from build123d import *

# Parameters (mm, degrees)
BRACKET_PROFILE_SKETCH_R   = 13
BRACKET_PROFILE_SKETCH_R_2 = 20
BRACKET_PROFILE_SKETCH_R_3 = 10
BRACKET_PROFILE_SKETCH_R_4 = 22
BRACKET_PLATE_12_5MM_DEPTH = 12.5
EDGE_FILLET_R15_R          = 15


with BuildPart() as part:
    # Bracket Profile Sketch → Bracket Plate 12.5mm (new body)
    with BuildSketch(Plane.XY):
        with BuildLine():
            Line((0, 119.020008006), (0, 0))
            Line((0, 0), (44, 0))
            Line((44, 0), (44, 22))
            ThreePointArc((44, 22), (58, 36), (72, 22))
            Line((72, 22), (72, 0))
            Line((72, 0), (96, 0))
            Line((96, 0), (96, 70))
            ThreePointArc((96, 70), (91.01229045, 88.819901149), (77.358490566, 102.699370682))
            ThreePointArc((77.358490566, 102.699370682), (71.968832717, 108.178108656), (70, 115.607017004))
            Line((70, 115.607017004), (70, 170))
            ThreePointArc((70, 170), (86.946326412, 200.621771092), (52, 198.717797887))
            ThreePointArc((52, 198.717797887), (38.977494473, 183.164838251), (20, 176))
            ThreePointArc((20, 176), (-10.194037026, 154.598119083), (0, 119.020008006))
        make_face()
        with Locations((20, 22)):
            Circle(BRACKET_PROFILE_SKETCH_R, mode=Mode.SUBTRACT)
        with Locations((20, 144)):
            Circle(BRACKET_PROFILE_SKETCH_R_2, mode=Mode.SUBTRACT)
        with Locations((70, 190)):
            Circle(BRACKET_PROFILE_SKETCH_R_3, mode=Mode.SUBTRACT)
        with Locations((58, 70)):
            Circle(BRACKET_PROFILE_SKETCH_R_4, mode=Mode.SUBTRACT)
    extrude(amount=BRACKET_PLATE_12_5MM_DEPTH)

    # Edge Fillet R15
    edge_fillet_r15_edges = [part.edges().sort_by_distance(p)[0] for p in [
        (70, 170, 6.25),
    ]]
    fillet(edge_fillet_r15_edges, radius=EDGE_FILLET_R15_R)


solid = part.part
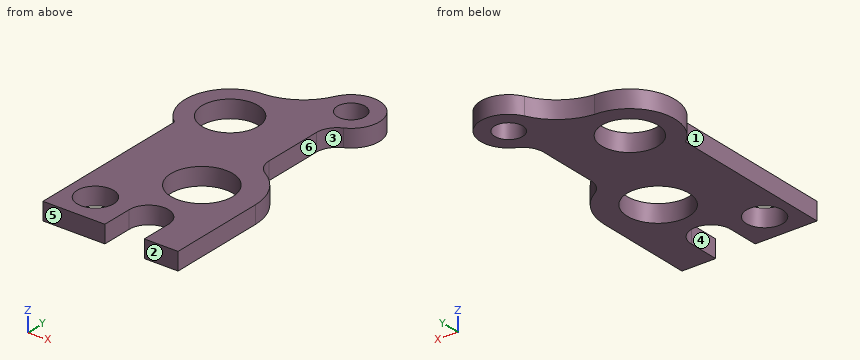
The model under review builds one solid part; all positions refer to its coordinate system, in mm. Face numbers are marked on the shaded views. A direction names the side the tool comes from. Give positions to 0.01 mm unless a question says otherwise; leave off trailing zeros. Order: outer loops, then holes, each group sorted by start corner. A loop starts at its lowest first (then second) coordinate and runs counter-clockwise, first axis right, second up. Notation, with made-up numbers: M 49,87 L 97,87 A9 ccw 97,99 Z; hole C -24,56 d2. An arc over 180 degrees is marked long. Answer in a Markdown table with one row per item. Add a question column.
1. Add section D-D on x = 24.5. State the section outline as (y, z) points.
2. Machinability: for the marked faces 4, 5 and 6, which of the approach directions +Z, -Z, +X, -X, +Y, -Y give a long, thin tool a straight path to every point of the face, cutting with its end or side? Answer none if there is none.
3. Mouldability with a two-part tool opening along Y and no side actions: class the marked faces 1, 2 and 3 as released by +Y, released by -Y, zero draft, split by the parting line, or undercut.
4. Add section C-C on x = 46.5. State the section outline as (y, z) points (3 decimals).
5. To check wall thickness, follow line 1 along Y through (x, z) = (20, 5.25); line 2 along Y through (x, z) = (29.5, 6.5); line 3 along X through (y, z) = (79, 6.75). State the ranges of each line that lie inside material, in increasing order.
6. Add section A-A on z = 5.75. State the section outline as (x, y) points, plus the area to 3 significant figures.
7. For pin 1 Ø6 at (y, z) = (130, 7.5) entering from +X; pin 2 Ø4 at (y, z) = (37, 10.5) entering from -X, all flat-tipped, find the tip position at first contact; note any pin that passes through.
8. Add section B-B on y = 144. State the section outline as (x, z) points, plus the area to 3 significant figures.
The answers:
| question | item | result |
|---|---|---|
| 1 | outline | M 0,0 L 9.8,0 L 9.8,12.5 L 0,12.5 Z; M 34.2,0 L 124.51,0 L 124.51,12.5 L 34.2,12.5 Z; M 163.49,0 L 176.73,0 L 176.73,12.5 L 163.49,12.5 Z |
| 2 | face 4 | +Z, -Z, -Y |
| 2 | face 5 | +Z, -Z, +X, -X, -Y |
| 2 | face 6 | +Z, -Z, +X |
| 3 | face 1 | zero draft |
| 3 | face 2 | released by -Y |
| 3 | face 3 | undercut |
| 4 | outline | M 29.984,0 L 51.245,0 L 51.245,12.5 L 29.984,12.5 Z; M 88.755,0 L 190.113,0 L 190.113,12.5 L 88.755,12.5 Z |
| 5 | line 1 | 0 to 9, 35 to 124, 164 to 176 |
| 5 | line 2 | 0 to 13.13, 30.87 to 126.4, 161.6 to 178.19 |
| 5 | line 3 | 0 to 37.93, 78.07 to 94.92 |
| 6 | outline | M 0,0 L 44,0 L 44,22 A14 cw 72,22 L 72,0 L 96,0 L 96,70 A38 ccw 77.36,102.7 A15 cw 70,115.61 L 70,158.38 A15 cw 78.57,171.93 A20 ccw long 52,198.72 A40 cw 20,176 A32 ccw 0,119.02 Z; hole C 20,144 d40; hole C 20,22 d26; hole C 58,70 d44; hole C 70,190 d20 |
| 6 | area | 12,100 mm2 |
| 7 | pin 1 | x = 70 |
| 7 | pin 2 | x = 0 |
| 8 | outline | M -12,0 L 0,0 L 0,12.5 L -12,12.5 Z; M 40,0 L 70,0 L 70,12.5 L 40,12.5 Z |
| 8 | area | 525 mm2 |
